Geometry check sheet. Reference: the model listing, model coordinates, mm. Round coordinates to 2 decimals unless told otherwise and drop trailing zeros. Return JSON: item names as keys, results as strings. Group by question number.
```python
from build123d import *

# Parameters (mm, degrees)
SKETCH1_W                   = 60
SKETCH1_H                   = 30
BOSS_EXTRUDE1_DEPTH         = 20
M6_TAPPED_HOLE1_D           = 5
M6_TAPPED_HOLE1_DEPTH       = 15
M6_TAPPED_HOLE1_CSINK_D     = 6.05
M6_TAPPED_HOLE1_CSINK_ANGLE = 90
M6_TAPPED_HOLE1_TIP         = 1.502151548


with BuildPart() as part:
    # Sketch1 → Boss-Extrude1 (new body)
    with BuildSketch(Plane.XY):
        with Locations((720, 45)):
            Rectangle(SKETCH1_W, SKETCH1_H)
    extrude(amount=BOSS_EXTRUDE1_DEPTH)

    # M6 Tapped Hole1
    with Locations(Plane.XY.offset(20)):
        with Locations((720, 45)):
            CounterSinkHole(M6_TAPPED_HOLE1_D / 2, M6_TAPPED_HOLE1_CSINK_D / 2, depth=M6_TAPPED_HOLE1_DEPTH, counter_sink_angle=M6_TAPPED_HOLE1_CSINK_ANGLE)
            with Locations((0, 0, -(M6_TAPPED_HOLE1_DEPTH + M6_TAPPED_HOLE1_TIP / 2))):  # 118° drill point
                Cone(0, M6_TAPPED_HOLE1_D / 2, M6_TAPPED_HOLE1_TIP, mode=Mode.SUBTRACT)


solid = part.part
```
Q1. Material ranges on line 1 along Y through (x, z) = (720, 13); line 2 along X through (y, z) = (45, 11); line 3 along X through (y, z) = (43, 10.5), recorded low to high.
Q2. Depth check by flat-ended pin: pin 1 Ø4.5 at (x, y) = (720, 45) entering from +Z. Enter the tip coordinate at first touch or a pass-through.
Q3. Release check for a two-part mould opening along Y. For faces 1 (the face through (717.69, 44.04, 12.14)), 2 (the face through (720, 30, 10)), 3 (the face through (719.566, 45.019, 3.759)), 4 (the face through (720, 60, 10)) record: +Y half, -Y half, draft (parallel to the pull), parting line (faces both ways), or undercut.
Geometry check:
{
 "1": {"line 1": "y = 30 to 42.5, 47.5 to 60", "line 2": "x = 690 to 717.5, 722.5 to 750", "line 3": "x = 690 to 718.5, 721.5 to 750"},
 "2": {"pin 1": "stops at z = 4.85"},
 "3": {"face 1": "undercut", "face 2": "-Y half", "face 3": "undercut", "face 4": "+Y half"}
}
